Check sheet for the modelled part. Datum: model origin and axes. Units: mm. A direction names the side the tool comes from. Give positions to 0.01 mm unless a question says otherwise; leave off trailing zeros. Order: outer loops, then holes, each group sorted by start corner. A loop starts at its lowest first (then second) coordinate and runs counter-clockwise, first axis right, second up.
from build123d import *

# Parameters (mm, degrees)
SKETCH_1_R          = 16
EXTRUDE_1_DEPTH     = 2
SKETCH_2_R          = 15
EXTRUDE_2_DEPTH     = 66
SKETCH_3_R          = 9
CUT_EXTRUDE_1_DEPTH = 72.665891469
SKETCH_5_R          = 11
CUT_EXTRUDE_2_DEPTH = 66
SKETCH_8_R          = 3
CUT_EXTRUDE_3_DEPTH = 10
SKETCH_9_W          = 1.3
SKETCH_9_H          = 0.7
CHAMFER_1_SIZE      = 0.5
SKETCH_10_W         = 0.5
SKETCH_10_H         = 1


with BuildPart() as part:
    # 草图1 → 凸台-拉伸1 (new body)
    with BuildSketch(Plane.XY):
        Circle(SKETCH_1_R)
    extrude(amount=EXTRUDE_1_DEPTH)

    # 草图2 → 凸台-拉伸2 (add)
    with BuildSketch(Plane.XY.offset(2)):
        Circle(SKETCH_2_R)
    extrude(amount=EXTRUDE_2_DEPTH)

    # 草图3 → 切除-拉伸1 (cut, through all)
    with BuildSketch(Plane(origin=(0, 0, 0), x_dir=(-1, 0, 0), z_dir=(0, 0, -1))):
        Circle(SKETCH_3_R)
    extrude(amount=-CUT_EXTRUDE_1_DEPTH, mode=Mode.SUBTRACT)

    # 草图5 → 切除-拉伸2 (cut)
    with BuildSketch(Plane.XY.offset(68)):
        Circle(SKETCH_5_R)
    extrude(amount=-CUT_EXTRUDE_2_DEPTH, mode=Mode.SUBTRACT)

    # 草图8 → 切除-拉伸3 (cut)
    with BuildSketch(Plane(origin=(0, 15, 0), x_dir=(1, 0, 0), z_dir=(0, 1, 0))):
        with Locations(Location((0, -32, 0), (0, 0, 270))):
            Circle(SKETCH_8_R)
    extrude(amount=-CUT_EXTRUDE_3_DEPTH, mode=Mode.SUBTRACT)

    # 草图9 → 切除-旋转1 (revolve, cut)
    with BuildSketch(Plane(origin=(0, 0, 0), x_dir=(0, 0, -1), z_dir=(1, 0, 0)), mode=Mode.PRIVATE) as cut_revolve_1_sk:
        with Locations((-52.55, 14.65)):
            Rectangle(SKETCH_9_W, SKETCH_9_H)
    revolve(cut_revolve_1_sk.sketch.rotate(Axis((0, 0, 68), (0, 0, -1)), 90), axis=Axis((0, 0, 68), (0, 0, -1)), mode=Mode.SUBTRACT)

    # 倒角1
    chamfer_1_edges = [part.edges().sort_by_distance(p)[0] for p in [
        (-16, 0, 0),
        (-15, 0, 68),
    ]]
    chamfer(chamfer_1_edges, length=CHAMFER_1_SIZE)

    # 草图10 → 切除-旋转2 (revolve, cut)
    with BuildSketch(Plane(origin=(0, 0, 0), x_dir=(1, 0, 0), z_dir=(0, 1, 0))):
        with Locations((-14.75, -2.5)):
            Rectangle(SKETCH_10_W, SKETCH_10_H)
    revolve(axis=Axis((0, 0, 0), (0, 0, 1)), mode=Mode.SUBTRACT)


solid = part.part
1) Material ranges on L1, parallel to Y at x = 0, z = 16; L2, parallel to Y at x = 0, z = 0.6; L3, parallel to Z at x = 0, y = 13.75, recorded low to high.
Recorded:
L1: y = -15 to -11, 11 to 15
L2: y = -16 to -9, 9 to 16
L3: z = 0 to 29, 35 to 68
2) Section check B-B, the plane z = 8.5. Record the cut outline in (x, y), then the cut area to 3 significant figures.
Recorded:
outline: circle Ø30 at (0, 0); hole circle Ø22 at (0, 0)
area: 327 mm2
3) Set-up check for faces 4 (the face through (-1.86, -14.18, 52.54)), 5 (the face through (-3.252, -14.643, 27.108)), 6 (the face through (3, 13, 32)): record each of +Z, -Z, +X, -X, +Y, -Y from which the full face is reachable in a straight line by a thin tool's end or side.
Recorded:
face 4: none
face 5: +Z
face 6: +Y
4) Depth check by flat-ended pin: pin 1 Ø1 at (y, z) = (-6, 29.5) entering from -X; pin 2 Ø12 at (y, z) = (12, 61) entering from -X; pin 3 Ø8 at (x, z) = (-10, 14.5) entering from +Y. Enter the tip coordinate at first touch or a pass-through.
Recorded:
pin 1: stops at x = -13.96
pin 2: stops at x = -13.75
pin 3: stops at y = 13.75
5) Draft check along Y on faces 1 (the face through (-14.985, 0.66, 60.25)), 2 (the face through (7, -7, 0)), 3 (the face through (-2.38, -10.74, 35.46)). Enter one of: +Y half, -Y half, draft (parallel to the pull), parting line (faces both ways), or undercut.
Recorded:
face 1: parting line
face 2: draft
face 3: undercut
6) Section check C-C, the plane z = 32. Record the cut outline in (x, y).
Recorded:
outline: (-3, 10.58) - (-3, 14.7) arc R15 ccw (long way) to (3, 14.7) - (3, 10.58) arc R11 cw (long way) to start
7) Section check A-A, the plane x = 0. State how many separate pieces and enclosed holes the cut face has, then the cut area to 3 significant figures.
Recorded:
separate pieces: 3
enclosed holes: 0
area: 529 mm2
